from build123d import *

# Parameters (mm, degrees)
SKETCH1_R           = 13
BOSS_EXTRUDE1_DEPTH = 10
SKETCH2_R           = 14
BOSS_EXTRUDE2_DEPTH = 26
SKETCH3_R           = 13
BOSS_EXTRUDE3_DEPTH = 10
SKETCH4_R           = 1.5
BOSS_EXTRUDE4_DEPTH = 10


with BuildPart() as part:
    # Sketch1 → Boss-Extrude1 (new body)
    with BuildSketch(Plane(origin=(0, 0, 0), x_dir=(1, 0, 0), z_dir=(0, 1, 0))):
        with Locations(Location((0, 0, 0), (0, 0, 270))):
            Circle(SKETCH1_R)
    extrude(amount=BOSS_EXTRUDE1_DEPTH)

    # Sketch2 → Boss-Extrude2 (add)
    with BuildSketch(Plane(origin=(0, 10, 0), x_dir=(1, 0, 0), z_dir=(0, 1, 0))):
        with Locations(Location((0, 0, 0), (0, 0, 90))):
            Circle(SKETCH2_R)
    extrude(amount=BOSS_EXTRUDE2_DEPTH)

    # Sketch3 → Boss-Extrude3 (add)
    with BuildSketch(Plane(origin=(0, 36, 0), x_dir=(1, 0, 0), z_dir=(0, 1, 0))):
        with Locations(Location((0, 0, 0), (0, 0, 270))):
            Circle(SKETCH3_R)
    extrude(amount=BOSS_EXTRUDE3_DEPTH)

    # Sketch4 → Boss-Extrude4 (add)
    with BuildSketch(Plane(origin=(0, 46, 0), x_dir=(1, 0, 0), z_dir=(0, 1, 0))):
        with Locations(Location((0, 0, 0), (0, 0, 270))):
            Circle(SKETCH4_R)
    extrude(amount=BOSS_EXTRUDE4_DEPTH)


solid = part.part
Work out the finished part from the listing and answer in its coordinate system (mm). A direction names the side the tool comes from. Coordinates: 2 decimals unless noted, no trailing zeros. Write each loop counter-clockwise with the first axis right and the second up, starting at its lowest first coordinate (ties: lowest second). Pieces come first, ordered by that corner, then holes. Notation, with made-up numbers: M 53,45 L 109,45 A14 cw 109,50 Z; hole C -33,7.25 d8. An arc over 180 degrees is marked long. Use one line per item in the form item = value. Start each with the question number.
1. A tool of negligible diameter and unlimited length cuts with its end or side. For faces 1 (the face through (9.3, 10, -9.3)), 2 (the face through (-7.91, 40.93, -10.316)), 3 (the face through (0, 0, 0)), from which of +Z, -Z, +X, -X, +Y, -Y can it reach the whole face along a straight path? Write none if from no direction.
2. The part is cut by section D-D (x = -9.75). Give the vertices of the cut face in (y, z), plus the area to 3 significant figures.
3. Each of these flat-tipped pins is pushed along its axis until it touches: P1, Ø2, axis at x = 6, z = 6.5, coming from the +Y side; P2, Ø5, axis at x = 9, y = 16, coming from the +Z side; P3, Ø8, axis at y = 22.5, z = -5.5, coming from the -X side; P4, Ø1, axis at x = 11, z = 11, coming from the +Y side. Where does it stop, or does it pass through?
4. The part is cut by section A-A (x = 0). Give the vertices of the cut face in (y, z).
5. Straight lines are drawn through the part: probe 1 along Y at (x, z) = (-10, -1); probe 2 along Z at (x, y) = (0.5, 18.5); probe 3 along X at (y, z) = (40, -8). For each, find the intervals that lie inside material, in ascending order. Write a range as from..to.
6. The part is cut by section C-C (y = 49.5). Give the vertices of the cut face in (x, z), plus the area to 3 significant figures.
7. The part is cut by section B-B (z = 0). Give the vertices of the cut face in (x, y).
Evaluation:
q1.face_1 = -Y
q1.face_2 = +Y
q1.face_3 = +Z, -Z, +X, -X, -Y
q2.outline = M 0,-8.6 L 10,-8.6 L 10,-10.05 L 36,-10.05 L 36,-8.6 L 46,-8.6 L 46,8.6 L 36,8.6 L 36,10.05 L 10,10.05 L 10,8.6 L 0,8.6 Z
q2.area = 866 mm^2
q3.P1 = 46
q3.P2 = 12.4
q3.P3 = -13.92
q3.P4 = through
q4.outline = M 0,-13 L 10,-13 L 10,-14 L 36,-14 L 36,-13 L 46,-13 L 46,-1.5 L 56,-1.5 L 56,1.5 L 46,1.5 L 46,13 L 36,13 L 36,14 L 10,14 L 10,13 L 0,13 Z
q5.probe_1 = 0..46
q5.probe_2 = -13.99..13.99
q5.probe_3 = -10.25..10.25
q6.outline = C 0,0 d3
q6.area = 7.07 mm^2
q7.outline = M -14,10 L -13,10 L -13,0 L 13,0 L 13,10 L 14,10 L 14,36 L 13,36 L 13,46 L 1.5,46 L 1.5,56 L -1.5,56 L -1.5,46 L -13,46 L -13,36 L -14,36 Z
